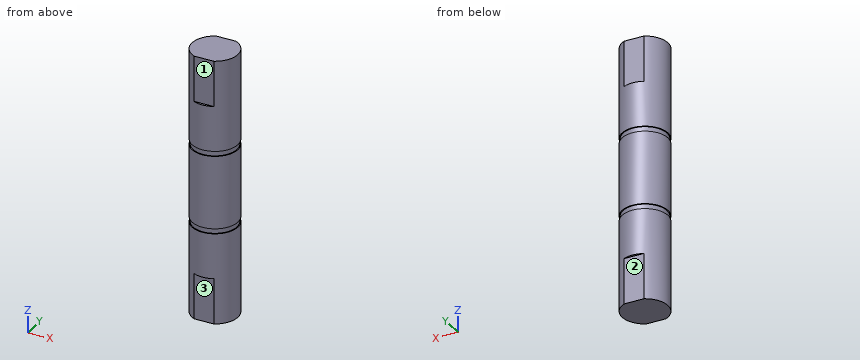
from build123d import *

# Parameters (mm, degrees)
SKETCH_1_R          = 5
EXTRUDE_1_DEPTH     = 29
CUT_EXTRUDE_START   = 1.1
SKETCH_3_R          = 5
SKETCH_3_R_2        = 4.8
CUT_EXTRUDE_2_DEPTH = 1.1
CUT_EXTRUDE_1_DEPTH = 10


with BuildPart() as part:
    # 草图1 → 凸台-拉伸1 (new, symmetric)
    with BuildSketch(Plane.XY):
        with Locations(Location((0, 0, 0), (0, 0, 180))):
            Circle(SKETCH_1_R)
    extrude(amount=EXTRUDE_1_DEPTH, both=True)

    # 草图3 → 切除-拉伸2 (cut)
    with BuildSketch(Plane.XY.offset(8).offset(CUT_EXTRUDE_START)):
        with Locations(Location((0, 0, 0), (0, 0, 180))):
            Circle(SKETCH_3_R)
        Circle(SKETCH_3_R_2, mode=Mode.SUBTRACT)
    cut_extrude_2 = extrude(amount=-CUT_EXTRUDE_2_DEPTH, mode=Mode.SUBTRACT)

    # 镜向2: 切除-拉伸2 across plane
    add(cut_extrude_2.mirror(Plane.XY), mode=Mode.SUBTRACT)

    # 草图2 → 切除-拉伸1 (cut)
    with BuildSketch(Plane.XY.offset(29)):
        with BuildLine():
            Line((-2.179449472, 4.5), (2.179449472, 4.5))
            ThreePointArc((2.179449472, 4.5), (0, 5), (-2.179449472, 4.5))
        make_face()
        with BuildLine():
            Line((-2.179449472, -4.5), (2.179449472, -4.5))
            ThreePointArc((2.179449472, -4.5), (0, -5), (-2.179449472, -4.5))
        make_face()
    cut_extrude_1 = extrude(amount=-CUT_EXTRUDE_1_DEPTH, mode=Mode.SUBTRACT)

    # 镜向1: 切除-拉伸1 across plane
    add(cut_extrude_1.mirror(Plane.XY), mode=Mode.SUBTRACT)


solid = part.part
Geometry: final body of the model. Coordinates: model frame, mm. Face numbers are marked on the shaded views. A direction names the side the tool comes from. Give positions to 0.01 mm unless a question says otherwise; leave off trailing zeros. Loops run counter-clockwise (first coordinate to the right, second up) from the corner with the lowest first, then second, coordinate; pieces in that order, holes last. Notation, with made-up numbers: M 59.5,79 L 77.5,79 A24 ccw 77.5,113 Z; hole C 39,18.5 d5. An arc over 180 degrees is marked long. Put each result on its own line as item: value.
1) Material intervals for L1, parallel to X at y = 0.25, z = 24; L2, parallel to Y at x = -0.25, z = -9; L3, parallel to X at y = 4.5, z = 14, sorted ascending. Write a range as from..to.
Computed values:
L1: x = -4.99..4.99
L2: y = -4.79..4.79
L3: x = -2.18..2.18
2) Cut plane D-D, the plane x = -3. Return the cut outline in (y, z).
Computed values:
outline: M -4,-29 L 4,-29 L 4,-9.1 L 3.75,-9.1 L 3.75,-8 L 4,-8 L 4,8 L 3.75,8 L 3.75,9.1 L 4,9.1 L 4,29 L -4,29 L -4,9.1 L -3.75,9.1 L -3.75,8 L -4,8 L -4,-8 L -3.75,-8 L -3.75,-9.1 L -4,-9.1 Z
3) Cut plane C-C, the plane y = -2.5. Return the cut outline in (x, z), plus the area to 3 significant figures.
Computed values:
outline: M -4.33,-29 L 4.33,-29 L 4.33,-9.1 L 4.1,-9.1 L 4.1,-8 L 4.33,-8 L 4.33,8 L 4.1,8 L 4.1,9.1 L 4.33,9.1 L 4.33,29 L -4.33,29 L -4.33,9.1 L -4.1,9.1 L -4.1,8 L -4.33,8 L -4.33,-8 L -4.1,-8 L -4.1,-9.1 L -4.33,-9.1 Z
area: 501 mm^2
4) First-contact query: P1, Ø1.5, axis at y = 1.5, z = -9, coming from the +X side; P2, Ø2, axis at y = 3.5, z = 0.5, coming from the -X side; P3, Ø5, axis at x = 0, z = 23.5, coming from the +Y side. Flat tips, straight axial feed; report the tip coordinate or a pass-through.
Computed values:
P1: stops at x = 4.94
P2: stops at x = -4.33
P3: stops at y = 4.5
5) Reachability of the marked faces 1, 2 and 3 from +Z, -Z, +X, -X, +Y, -Y: full face, straight path, thin tool, end or side. Return the list, or none.
Computed values:
face 1: +Z, +X, -X, -Y
face 2: -Z, +X, -X, +Y
face 3: -Z, +X, -X, -Y
6) Cut plane A-A, the plane x = 0. Return the cut outline in (y, z), plus the area to 3 significant figures.
Computed values:
outline: M -5,-19 L -4.5,-19 L -4.5,-29 L 4.5,-29 L 4.5,-19 L 5,-19 L 5,-9.1 L 4.8,-9.1 L 4.8,-8 L 5,-8 L 5,8 L 4.8,8 L 4.8,9.1 L 5,9.1 L 5,19 L 4.5,19 L 4.5,29 L -4.5,29 L -4.5,19 L -5,19 L -5,9.1 L -4.8,9.1 L -4.8,8 L -5,8 L -5,-8 L -4.8,-8 L -4.8,-9.1 L -5,-9.1 Z
area: 559 mm^2
7) Cut plane B-B, the plane z = -17. Return the cut outline in (x, y), plus the area to 3 significant figures.
Computed values:
outline: C 0,0 d10
area: 78.5 mm^2
